Work out the finished part from the listing and answer in its coordinate system (mm). Face numbers are marked on the shaded views. Round coordinates to 2 decimals unless told otherwise and drop trailing zeros. Write each loop counter-clockwise with the first axis right and the second up, starting at its lowest first coordinate (ties: lowest second). Pieces come first, ordered by that corner, then holes. Notation, with made-up numbers: M 22,-37.5 L 67,-37.5 A20 ccw 67,-21.5 Z; hole C 51.25,33 d11. An arc over 180 degrees is marked long. Answer in a Markdown table with one row per item.
```python
from build123d import *

# Parameters (mm, degrees)
SKETCH_1_W          = 70
SKETCH_1_H          = 40
EXTRUDE_1_DEPTH     = 5
HOLE_WIZARD_M10_1_D = 11
FILLET_1_R          = 5


with BuildPart() as part:
    # 草图1 → 凸台-拉伸1 (new, symmetric)
    with BuildSketch(Plane(origin=(0, 0, 0), x_dir=(1, 0, 0), z_dir=(0, 1, 0))):
        Rectangle(SKETCH_1_W, SKETCH_1_H)
    extrude(amount=EXTRUDE_1_DEPTH, both=True)

    # M10 间隙孔1 (through all)
    with Locations(Plane(origin=(0, 5, 0), x_dir=(1, 0, 0), z_dir=(0, 1, 0))):
        with Locations((-17.5, 12.5), (17.5, 12.5), (17.5, -12.5), (-17.5, -12.5)):
            Hole(HOLE_WIZARD_M10_1_D / 2)

    # 圆角1
    fillet_1_edges = [part.edges().sort_by_distance(p)[0] for p in [
        (35, 0, 20),
        (-35, 0, 20),
        (-35, 0, -20),
        (35, 0, -20),
    ]]
    fillet(fillet_1_edges, radius=FILLET_1_R)


solid = part.part
```
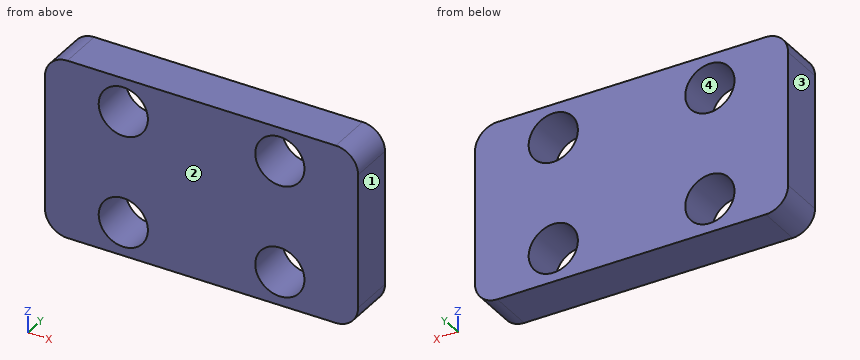
1. The part is cut by section A-A (x = 17.5). Determine the outline of the cut face in (y, z), plus the area to 3 significant figures.
Calculated:
| item | result |
|---|---|
| outline | M -5,-20 L 5,-20 L 5,-18 L -5,-18 Z; M -5,-7 L 5,-7 L 5,7 L -5,7 Z; M -5,18 L 5,18 L 5,20 L -5,20 Z |
| area | 180 mm² |
2. The part is cut by section C-C (y = -2). Determine the outline of the cut face in (x, z), plus the area to 3 significant figures.
Calculated:
| item | result |
|---|---|
| outline | M -35,-15 A5 ccw -30,-20 L 30,-20 A5 ccw 35,-15 L 35,15 A5 ccw 30,20 L -30,20 A5 ccw -35,15 Z; hole C -17.5,-12.5 d11; hole C -17.5,12.5 d11; hole C 17.5,-12.5 d11; hole C 17.5,12.5 d11 |
| area | 2,400 mm² |
3. The part is cut by section B-B (z = -12.5). Determine the outline of the cut face in (x, y), plus the area to 3 significant figures.
Calculated:
| item | result |
|---|---|
| outline | M -35,-5 L -23,-5 L -23,5 L -35,5 Z; M -12,-5 L 12,-5 L 12,5 L -12,5 Z; M 23,-5 L 35,-5 L 35,5 L 23,5 Z |
| area | 480 mm² |
4. Consider line 1 along Z through (x, y) = (17.5, -2); line 2 along Z through (x, y) = (15.5, 3.25); line 3 along X through (y, z) = (0.5, 10). Determine where each line is inside the solid, lowest interval first. Write a range as from..to.
Calculated:
| item | result |
|---|---|
| line 1 | z = -20..-18, -7..7, 18..20 |
| line 2 | z = -20..-17.62, -7.38..7.38, 17.62..20 |
| line 3 | x = -35..-22.4, -12.6..12.6, 22.4..35 |
5. Determine the mould class of the marked faces 1, 2, 3 and 4 for opening direction X: released by +X, released by -X, zero draft, split by the parting line, or undercut.
Calculated:
| item | result |
|---|---|
| face 1 | released by +X |
| face 2 | zero draft |
| face 3 | released by -X |
| face 4 | undercut |
